from build123d import *

# Parameters (mm, degrees)
MM_1_D              = 2.2
MM_1_DEPTH          = 7.1
MM_1_TIP            = 0.660946681
SKETCH_7_R          = 2.5
SKETCH_7_R_2        = 1.5
CUT_EXTRUDE_1_DEPTH = 5
SKETCH_8_R          = 1.5
CUT_EXTRUDE_2_DEPTH = 5


with BuildPart() as part:
    # 草图1 → 旋转1 (revolve)
    with BuildSketch(Plane.XY, mode=Mode.PRIVATE) as revolve_1_sk:
        Polygon((0, 0), (12.45, 0), (12.45, 1.295), (11.1546, 1.295), (11.1546, 3.708), (12.45, 3.708), (12.45, 5), (16, 5), (16, 7), (0, 7), align=None)
    revolve(revolve_1_sk.sketch.rotate(Axis((0, 7, 0), (0, -1, 0)), 90), axis=Axis((0, 7, 0), (0, -1, 0)))

    # 大小mm 暗销孔1
    with Locations(Plane(origin=(0, 7, 0), x_dir=(1, 0, 0), z_dir=(0, 1, 0))):
        with Locations((-10.076271632, -10.076271632), (-10.076271632, 10.076271632), (10.076271632, 10.076271632), (10.076271632, -10.076271632)):
            Hole(MM_1_D / 2, depth=MM_1_DEPTH)
            with Locations((0, 0, -(MM_1_DEPTH + MM_1_TIP / 2))):  # 118° drill point
                Cone(0, MM_1_D / 2, MM_1_TIP, mode=Mode.SUBTRACT)

    # 草图7 → 切除-拉伸1 (cut)
    with BuildSketch(Plane.XZ):
        with Locations(Location((-9, 0, 0), (0, 0, 270))):
            Circle(SKETCH_7_R)
        with Locations(Location((9, 0, 0), (0, 0, 270))):
            Circle(SKETCH_7_R)
        with Locations(Location((0, -7, 0), (0, 0, 270))):
            Circle(SKETCH_7_R_2)
        with Locations(Location((0, 7, 0), (0, 0, 270))):
            Circle(SKETCH_7_R_2)
    extrude(amount=-CUT_EXTRUDE_1_DEPTH, mode=Mode.SUBTRACT)

    # 草图8 → 切除-拉伸2 (cut)
    with BuildSketch(Plane.XZ.offset(-5)):
        with Locations(Location((0, 7, 0), (0, 0, 270))):
            Circle(SKETCH_8_R)
        with Locations(Location((0, -7, 0), (0, 0, 270))):
            Circle(SKETCH_8_R)
    extrude(amount=-CUT_EXTRUDE_2_DEPTH, mode=Mode.SUBTRACT)


solid = part.part
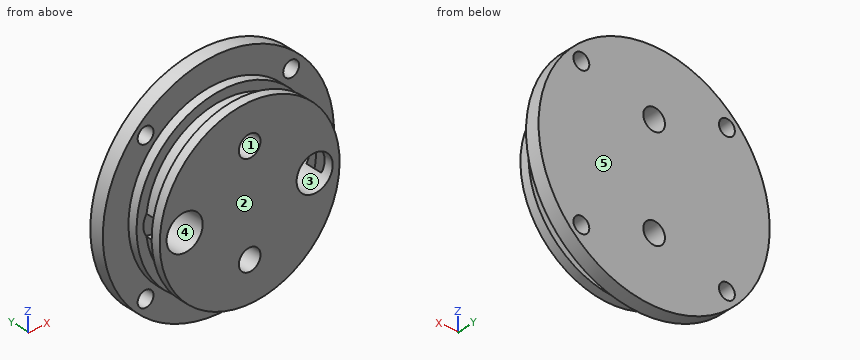
Verification items for the finished model (mm, model axes). Face numbers are marked on the shaded views. A direction names the side the tool comes from. Coordinates: 2 decimals unless noted, no trailing zeros. Loops run counter-clockwise (first coordinate to the right, second up) from the corner with the lowest first, then second, coordinate; pieces in that order, holes last. Notation, with made-up numbers: M 69,3.5 L 128,3.5 A12 cw 128,20.5 Z; hole C 37.25,55.25 d6. An arc over 180 degrees is marked long. One line per item, written item: value.
1. Section check B-B on z = 0. Record the cut outline in (x, y) (3 decimals), plus the area to 3 significant figures.
Answers follow:
outline: M -16,5 L -12.45,5 L -12.45,3.708 L -11.5,3.708 L -11.5,5 L -6.5,5 L -6.5,0 L 6.5,0 L 6.5,5 L 11.5,5 L 11.5,3.708 L 12.45,3.708 L 12.45,5 L 16,5 L 16,7 L -16,7 Z; M -12.45,0 L -11.5,0 L -11.5,1.295 L -12.45,1.295 Z; M 11.5,0 L 12.45,0 L 12.45,1.295 L 11.5,1.295 Z
area: 134 mm^2
2. Section check A-A on x = 0. Record the cut outline in (y, z) (3 decimals), plus the area to 3 significant figures.
Answers follow:
outline: M 0,-12.45 L 1.295,-12.45 L 1.295,-11.155 L 3.708,-11.155 L 3.708,-12.45 L 5,-12.45 L 5,-16 L 7,-16 L 7,-8.5 L 0,-8.5 Z; M 0,-5.5 L 7,-5.5 L 7,5.5 L 0,5.5 Z; M 0,8.5 L 7,8.5 L 7,16 L 5,16 L 5,12.45 L 3.708,12.45 L 3.708,11.155 L 1.295,11.155 L 1.295,12.45 L 0,12.45 Z
area: 140 mm^2
3. Section check D-D on y = 6. Record the cut outline in (x, z), plus the area to 3 significant figures.
Answers follow:
outline: C 0,0 d32; hole C -10.08,-10.08 d2.2; hole C -10.08,10.08 d2.2; hole C 0,-7 d3; hole C 0,7 d3; hole C 10.08,-10.08 d2.2; hole C 10.08,10.08 d2.2
area: 775 mm^2
4. Set-up check for the marked faces 4 and 5: record each of +Z, -Z, +X, -X, +Y, -Y from which the full face is reachable in a straight line by a thin tool's end or side.
Answers follow:
face 4: -Y
face 5: +Z, -Z, +X, -X, +Y
5. Material ranges on line 1 along X through (y, z) = (1.5, -2); line 2 along Y through (x, z) = (-11, 5.5) (3 decimals); line 3 along Z through (x, y) = (1, 4.25), recorded low to high. Write a range as from..to.
Answers follow:
line 1: -10.97..-10.5, -7.5..7.5, 10.5..10.97
line 2: 0..1.295, 3.708..7
line 3: -12.41..-8.12, -5.88..5.88, 8.12..12.41
6. Gauge pin test, flat ends, axial feed: P1, Ø2.5, axis at x = 10, z = 1, coming from the -Y side; P2, Ø4.5, axis at x = 9, z = 0, coming from the -Y side; P3, Ø2, axis at x = -10.08, z = -10.08, coming from the +Y side. Record the tip position at first contact, or that the pin passes through.
Answers follow:
P1: y = 0
P2: y = 5
P3: through
7. Section check C-C on z = -7. Record the cut outline in (x, y) (1 decimal), plus the area to 3 significant figures.
Answers follow:
outline: M -14.4,5 L -10.3,5 L -10.3,3.7 L -8.7,3.7 L -8.7,1.3 L -10.3,1.3 L -10.3,0 L -1.5,0 L -1.5,7 L -14.4,7 Z; M 1.5,0 L 10.3,0 L 10.3,1.3 L 8.7,1.3 L 8.7,3.7 L 10.3,3.7 L 10.3,5 L 14.4,5 L 14.4,7 L 1.5,7 Z
area: 132 mm^2
8. Mould release check, pull along Z, two halves, no side actions. Record for the marked faces 1, 2 and 3: pulls with the +Z half, pulls with the -Z half, needs draft (parallel to the pull), parting line crosses it, or undercut.
Answers follow:
face 1: undercut
face 2: needs draft
face 3: undercut
